from build123d import *

# Parameters (mm, degrees)
BASE_BLOCK_SKETCH_W       = 72
BASE_BLOCK_SKETCH_H       = 90
BASE_BLOCK_90X72X36_DEPTH = 18
ARC_RECESS_SKETCH_R       = 30
ARC_RECESS_60_DEPTH       = 12
BORE_24_DEPTH             = 117.653332571
RECESS_RELIEF_SKETCH_R    = 12
RECESS_RELIEF_CUT_DEPTH   = 118.728501222
BOTTOM_GROOVE_SKETCH_W    = 50
BOTTOM_GROOVE_SKETCH_H    = 6
BOTTOM_GROOVE_6X50_DEPTH  = 121.747670785
FORK_ARM_DEPTH            = 72
FORK_SLOT_24_DEPTH        = 190.67867566


with BuildPart() as part:
    # Base Block Sketch → Base Block 90x72x36 (new, symmetric)
    with BuildSketch(Plane.XY):
        with Locations((36, 45)):
            Rectangle(BASE_BLOCK_SKETCH_W, BASE_BLOCK_SKETCH_H)
    extrude(amount=BASE_BLOCK_90X72X36_DEPTH, both=True)

    # Arc Recess Sketch → Arc Recess Ø60 (cut)
    with BuildSketch(Plane.XY.offset(18)):
        with Locations((36, 45)):
            Circle(ARC_RECESS_SKETCH_R)
    extrude(amount=-ARC_RECESS_60_DEPTH, mode=Mode.SUBTRACT)

    # Bore Sketch → Bore Ø24 (cut, through all)
    with BuildSketch(Plane(origin=(72, 0, 0), x_dir=(0, 0, -1), z_dir=(1, 0, 0))):
        Polygon((-18, 66), (-6, 66), (-6, 45), (-6, 30), (-18, 30), align=None)
    extrude(amount=-BORE_24_DEPTH, mode=Mode.SUBTRACT)

    # Recess Relief Sketch → Recess Relief Cut (cut, through all)
    with BuildSketch(Plane.XY.offset(6)):
        with Locations((36, 45)):
            Circle(RECESS_RELIEF_SKETCH_R)
    extrude(amount=-RECESS_RELIEF_CUT_DEPTH, mode=Mode.SUBTRACT)

    # Bottom Groove Sketch → Bottom Groove 6x50 (cut, through all)
    with BuildSketch(Plane.XY.offset(18)):
        with Locations((47, 3)):
            Rectangle(BOTTOM_GROOVE_SKETCH_W, BOTTOM_GROOVE_SKETCH_H)
    extrude(amount=-BOTTOM_GROOVE_6X50_DEPTH, mode=Mode.SUBTRACT)

    # Fork Arm Sketch → Fork Arm (add)
    with BuildSketch(Plane(origin=(72, 0, 0), x_dir=(0, 0, -1), z_dir=(1, 0, 0))):
        Polygon((18, 6), (90, 6), (90, 0), (163, 0), (163, 25), (18, 25), align=None)
    extrude(amount=-FORK_ARM_DEPTH)

    # Fork Slot Sketch → Fork Slot 24 (cut, through all)
    with BuildSketch(Plane(origin=(0, 25, 0), x_dir=(1, 0, 0), z_dir=(0, 1, 0))):
        with BuildLine():
            Line((48, 163), (48, 113))
            ThreePointArc((48, 113), (36, 101), (24, 113))
            Line((24, 113), (24, 163))
            Line((24, 163), (48, 163))
        make_face()
    extrude(amount=-FORK_SLOT_24_DEPTH, mode=Mode.SUBTRACT)


solid = part.part
Part model, mm, in its own coordinate system. A direction names the side the tool comes from. Round coordinates to 2 decimals unless told otherwise and drop trailing zeros. Write each loop counter-clockwise with the first axis right and the second up, starting at its lowest first coordinate (ties: lowest second). Pieces come first, ordered by that corner, then holes. Notation, with made-up numbers: (52, -9) - (96, -9) arc R21 cw to (96, 29) - close; hole circle Ø3 at (51, 39.5). An arc over 180 degrees is marked (long way). Use CSV: the item, a comma, the result in double quotes.
Item 1: Flat gauge pins, fed straight in: P1, Ø21.5, axis at x = 34, z = -92.5, coming from the +Y side; P2, Ø8, axis at x = 29.5, z = -51.5, coming from the -Y side; P3, Ø3, axis at x = 50, y = 3.5, coming from the +Z side. Where does each tip first touch, or does it go through?
Results list:
P1,"stops at y = 25"
P2,"stops at y = 6"
P3,"stops at z = -90"
Item 2: Slice it at A-A, the plane y = 45. Write the cut outline in (x, z), then the cut area to 3 significant figures.
Results list:
outline,"(0, -18) - (24, -18) - (24, 6) - (0, 6) - close; (48, -18) - (72, -18) - (72, 6) - (48, 6) - close"
area,"1,150 mm²"
Item 3: Slice it at D-D, the plane x = 6.5. Write the cut outline in (y, z).
Results list:
outline,"(0, -163) - (25, -163) - (25, -18) - (90, -18) - (90, 18) - (66, 18) - (66, 6) - (30, 6) - (30, 18) - (0, 18) - (0, -18) - (6, -18) - (6, -90) - (0, -90) - close"
Item 4: Slice it at C-C, the plane z = -7.5. Write the cut outline in (x, y).
Results list:
outline,"(0, 0) - (22, 0) - (22, 6) - (72, 6) - (72, 90) - (0, 90) - close; hole circle Ø24 at (36, 45)"
Item 5: Tool access for faces 5 (the cylindrical face through (36, 15, 12)), 6 (the flat face through (67, 30, 12)), 7 (the flat face through (22, 3, 0)), 8 (the flat face through (35, 58, -18)): list every direction of +Z, -Z, +X, -X, +Y, -Y with a clear straight run to the whole face (end or side of a thin tool).
Results list:
face 5,"+Z"
face 6,"+Z, +X, -X"
face 7,"+Z, +X, -Y"
face 8,"-Z, +X, -X, +Y"
Item 6: Slice it at B-B, the plane z = -127.5. Write the cut outline in (x, y), then the cut area to 3 significant figures.
Results list:
outline,"(0, 0) - (24, 0) - (24, 25) - (0, 25) - close; (48, 0) - (72, 0) - (72, 25) - (48, 25) - close"
area,"1,200 mm²"
Item 7: Wall check: L1, parallel to Y at x = 36, z = 0.25; L2, parallel to Y at x = 37, z = -72; L3, parallel to Z at x = 18, y = 33. Give the ranges that are in metal, low to high.
Results list:
L1,"y = 6 to 33, 57 to 90"
L2,"y = 6 to 25"
L3,"z = -18 to 6"
Item 8: Pull direction Z, two halves, no side cores. Call faces 1 (the flat face through (5, 30, 12)), 2 (the flat face through (37, 6, -35)), 3 (the flat face through (37, 3, -90)), 4 (the flat face through (37, 58, 6)): pulls with the +Z half, pulls with the -Z half, needs draft (parallel to the pull), parting line crosses it, or undercut.
Results list:
face 1,"needs draft"
face 2,"undercut"
face 3,"undercut"
face 4,"pulls with the +Z half"
